from build123d import *

# Parameters (mm, degrees)
SKETCH_1_R              = 22.5
EXTRUDE_1_DEPTH         = 250
SKETCH_2_R              = 15
CUT_EXTRUDE_1_DEPTH     = 200
CUT_EXTRUDE2_DEPTH      = 210
CUT_EXTRUDE2_DEPTH_BACK = 210
SKETCH_3_R              = 12.5
SKETCH_4_R              = 53.120468805
CUT_EXTRUDE3_DEPTH      = 20
CHAMFER1_SIZE           = 10
CHAMFER2_SIZE           = 3
FILLET1_R               = 10


with BuildPart() as part:
    # 草图1 → 凸台-拉伸1 (new body)
    with BuildSketch(Plane(origin=(0, 0, 0), x_dir=(1, 0, 0), z_dir=(0, 1, 0))):
        with Locations(Location((0, 0, 0), (0, 0, 270))):
            Circle(SKETCH_1_R)
    extrude(amount=EXTRUDE_1_DEPTH)

    # 草图2 → 切除-拉伸1 (cut)
    with BuildSketch(Plane(origin=(0, 250, 0), x_dir=(1, 0, 0), z_dir=(0, 1, 0))):
        with Locations(Location((0, 0, 0), (0, 0, 270))):
            Circle(SKETCH_2_R)
    extrude(amount=-CUT_EXTRUDE_1_DEPTH, mode=Mode.SUBTRACT)

    # 草图3 → Cut-Extrude2 (cut, two sides: drawn at the far end of the back side and taken through both)
    with BuildSketch(Plane.XY.offset(-CUT_EXTRUDE2_DEPTH_BACK)):
        with Locations(Location((0, 30, 0), (0, 0, 90))):
            Circle(SKETCH_3_R)
    extrude(amount=CUT_EXTRUDE2_DEPTH + CUT_EXTRUDE2_DEPTH_BACK, mode=Mode.SUBTRACT)

    # 草图4 → Cut-Extrude3 (cut)
    with BuildSketch(Plane(origin=(0, 250, 0), x_dir=(1, 0, 0), z_dir=(0, 1, 0))):
        Circle(SKETCH_4_R)
    extrude(amount=-CUT_EXTRUDE3_DEPTH, mode=Mode.SUBTRACT)

    # Chamfer1
    chamfer1_edges = [part.edges().sort_by_distance(p)[0] for p in [
        (0, 0, -22.5),
    ]]
    chamfer(chamfer1_edges, length=CHAMFER1_SIZE)

    # Chamfer2
    chamfer2_edges = [part.edges().sort_by_distance(p)[0] for p in [
        (0, 230, -22.5),
    ]]
    chamfer(chamfer2_edges, length=CHAMFER2_SIZE)

    # Fillet1
    fillet1_edges = [part.edges().sort_by_distance(p)[0] for p in [
        (0, 10, -22.5),
    ]]
    fillet(fillet1_edges, radius=FILLET1_R)


solid = part.part
The model under review builds one solid part; all positions refer to its coordinate system, in mm. A direction names the side the tool comes from. Round coordinates to 2 decimals unless told otherwise and drop trailing zeros. Loops run counter-clockwise (first coordinate to the right, second up) from the corner with the lowest first, then second, coordinate; pieces in that order, holes last. Notation, with made-up numbers: (-11, -11.5) -> (38, -11.5) arc R35 cw to (38, 27.5) -> close; hole circle Ø7 at (6.5, 24.25). An arc over 180 degrees is marked (long way). Write item = value, one per line. Start each with the question number.
Item 1: Take a section at A-A on y = 87.5. Give the boundary of the cut face in (x, z).
Item 2: Insertion check: pin 1 (3 mm diameter, centred on y = 193.5, z = -5, fed in from -X); pin 2 (6 mm diameter, centred on y = 167, z = -9.5, fed in from -X); pin 3 (4 mm diameter, centred on y = 143.5, z = 6, fed in from +X). Each pin has a flat end and moves straight along its axis. Give the tip position at first contact, or say it passes through.
Item 3: Mouldability with a two-part tool opening along X and no side actions: class faces 3 (the flat face through (0, 50, 0)), 4 (the conical face through (17.43, 229.85, 9.07)), 5 (the flat face through (10, 230, 11.5)) as released by +X, released by -X, zero draft, split by the parting line, or undercut.
Item 4: To check wall thickness, follow L1, parallel to X at y = 113.5, z = 0; L2, parallel to X at y = 30, z = 6; L3, parallel to Z at x = -11, y = 98. State the ranges of each line that lie inside material, in increasing order.
Item 5: For faces 1 (the flat face through (0, 0, 0)), 2 (the cylindrical face through (0.66, 141.26, -14.985)), list the 3-axis set-ups (+Z, -Z, +X, -X, +Y, -Y) from which the entire face can be reached by the end or side of a thin tool; tool diameter is ignored.
Item 6: Take a section at B-B on y = 30. Give the boundary of the cut face in (x, z), plus the area to 3 significant figures.
Result:
q1.outline = circle Ø45 at (0, 0); hole circle Ø30 at (0, 0)
q2.pin_1 = -22.23
q2.pin_2 = -21.54
q2.pin_3 = 22.14
q3.face_3 = undercut
q3.face_4 = split by the parting line
q3.face_5 = zero draft
q4.L1 = -22.5 to -15, 15 to 22.5
q4.L2 = -21.69 to -12.5, 12.5 to 21.69
q4.L3 = -19.63 to -10.2, 10.2 to 19.63
q5.face_1 = +Z, -Z, +X, -X, -Y
q5.face_2 = +Y
q6.outline = (-12.5, -18.71) -> (-12.5, 18.71) arc R22.5 ccw to start; (12.5, -18.71) arc R22.5 ccw to (12.5, 18.71) -> close
q6.area = 526 mm²
